Input: dimensioned drawing with shaded views. Units: mm. Origin: part minimum x, y, z. Round coordinates to 2 decimals unless told otherwise and drop trailing zeros. Loops run counter-clockwise (first coordinate to the right, second up) from the corner with the lowest first, then second, coordinate; pieces in that order, holes last. Notation, with made-up numbers: (58, 50) -> (97, 50) arc R26 ccw to (97, 78) -> close; hole circle Ø2 at (19.5, 6.25). An arc over 180 degrees is marked (long way). Answer as a JSON object with one key per item and string values.
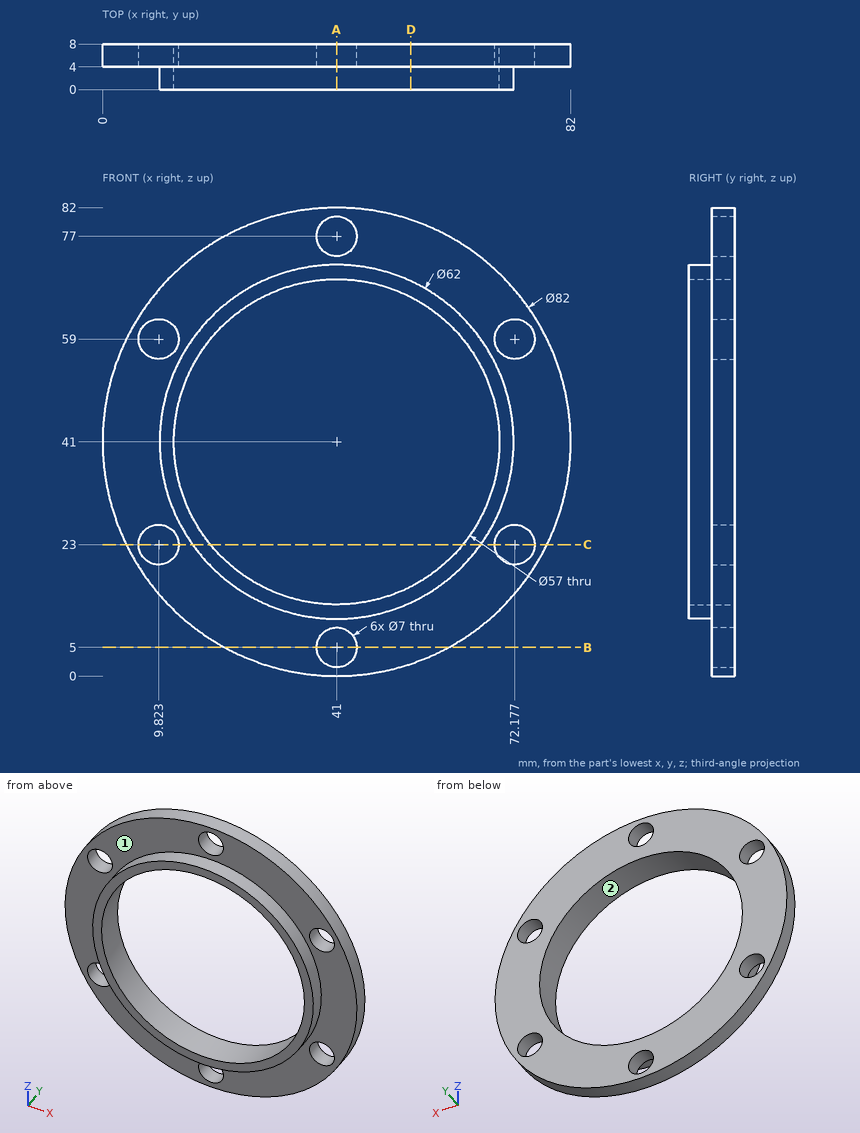
1) Section C-C, the plane z = 23. Output: boundary loops of the cut face in (x, y), plus the area to 3 significant figures.
Output:
{"outline": "(4.16, 4) -> (6.32, 4) -> (6.32, 8) -> (4.16, 8) -> close; (13.32, 4) -> (15.76, 4) -> (15.76, 0) -> (18.9, 0) -> (18.9, 8) -> (13.32, 8) -> close; (63.1, 0) -> (66.24, 0) -> (66.24, 4) -> (68.68, 4) -> (68.68, 8) -> (63.1, 8) -> close; (75.68, 4) -> (77.84, 4) -> (77.84, 8) -> (75.68, 8) -> close", "area": "87.1 mm^2"}
2) Contact query for a flat-ended pin moving along its axis: P1, Ø3, axis at y = 3.5, z = 30.5, coming from the -X side. Output: stop coordinate, or through.
Output:
{"P1": "stops at x = 1.02"}
3) Section D-D, the plane x = 54. Output: boundary loops of the cut face in (y, z), plus the area to 3 significant figures.
Output:
{"outline": "(0, 12.86) -> (4, 12.86) -> (4, 2.12) -> (8, 2.12) -> (8, 15.64) -> (0, 15.64) -> close; (0, 66.36) -> (8, 66.36) -> (8, 79.88) -> (4, 79.88) -> (4, 69.14) -> (0, 69.14) -> close", "area": "130 mm^2"}
4) Section A-A, the plane x = 41. Output: boundary loops of the cut face in (y, z).
Output:
{"outline": "(0, 10) -> (4, 10) -> (4, 8.5) -> (8, 8.5) -> (8, 12.5) -> (0, 12.5) -> close; (0, 69.5) -> (8, 69.5) -> (8, 73.5) -> (4, 73.5) -> (4, 72) -> (0, 72) -> close; (4, 0) -> (8, 0) -> (8, 1.5) -> (4, 1.5) -> close; (4, 80.5) -> (8, 80.5) -> (8, 82) -> (4, 82) -> close"}
5) Ray query, probe 1 along X at (y, z) = (5.4, 23); probe 2 along X at (y, z) = (3.5, 40.5); probe 3 along Z at (x, y) = (8, 5). Return the intervals inside material, ascending.
Output:
{"probe 1": "x = 4.16 to 6.32, 13.32 to 18.9, 63.1 to 68.68, 75.68 to 77.84", "probe 2": "x = 10 to 12.5, 69.5 to 72", "probe 3": "z = 16.67 to 20.01, 25.99 to 56.01, 61.99 to 65.33"}
6) Draft query along X for the marked faces 1 and 2. Return one class per face: +X half, -X half, draft (parallel to the pull), parting line (faces both ways), or undercut.
Output:
{"face 1": "draft", "face 2": "undercut"}
7) Section B-B, the plane z = 5. Output: boundary loops of the cut face in (x, y), plus the area to 3 significant figures.
Output:
{"outline": "(21.38, 4) -> (37.5, 4) -> (37.5, 8) -> (21.38, 8) -> close; (44.5, 4) -> (60.62, 4) -> (60.62, 8) -> (44.5, 8) -> close", "area": "129 mm^2"}
